Check sheet for the modelled part. Datum: model origin and axes. Units: mm. A direction names the side the tool comes from. Coordinates: 2 decimals unless noted, no trailing zeros. Write each loop counter-clockwise with the first axis right and the second up, starting at its lowest first coordinate (ties: lowest second). Pieces come first, ordered by that corner, then holes. Notation, with made-up numbers: (81, -8) -> (115, -8) arc R17 cw to (115, 3) -> close; hole circle Ø8 at (0, 4.5). An arc over 180 degrees is marked (long way). One line per item, written item: value. Start each with the question number.
1) Sectioned sample at A-A on x = -3. Enter the section's corners in (y, z).
2) Sectioned sample at B-B on y = 15.5. Enter the section's corners in (x, z).
3) Sectioned sample at D-D on y = -17.5. Enter the section's corners in (x, z).
4) Draft check along X on faces 5 (the flat face through (12, 23, 0)), 6 (the flat face through (0.18, -22.24, 6.92)), 7 (the flat face through (0, -21.5, 8)). Enter one of: +X half, -X half, draft (parallel to the pull), parting line (faces both ways), or undercut.
5) Scan lines: line 1 along Y through (x, z) = (1, 15); line 2 along Z through (x, y) = (0, 16); line 3 along Y through (x, z) = (-5.75, 10.75). Record each from-to range of solid material in increasing order. Write a range as [from, to].
6) Set-up check for faces 1 (the flat face through (0, 4, 3)), 2 (the flat face through (8.25, 16, -1)), 3 (the flat face through (0, -11, 14)), 4 (the cylindrical face through (10.288, -16.215, 5.296)): record each of +Z, -Z, +X, -X, +Y, -Y from which the full face is reachable in a straight line by a thin tool's end or side.
7) Gauge pin test, flat ends, axial feed: P1, Ø5, axis at x = -7.5, z = -0.5, coming from the -Y side; P2, Ø2, axis at x = 0, y = -17, coming from the -Z side; P3, Ø6, axis at x = -4.5, z = 12.5, coming from the +Y side; P4, Ø6.5, axis at x = 0, y = -18, coming from the -Z side. Record the tip position at first contact, or that the pin passes through.
8) Sectioned sample at C-C on z = 14. Enter the section's corners in (x, y), plus the area to 3 significant figures.
```python
from build123d import *

# Parameters (mm, degrees)
SKETCH1_W             = 25
SKETCH1_H             = 48
BOSS_EXTRUDE1_DEPTH   = 4
SKETCH5_W             = 25
SKETCH5_H             = 24
BOSS_EXTRUDE3_DEPTH   = 13
SKETCH6_W             = 20
SKETCH6_H             = 40
CUT_EXTRUDE1_DEPTH    = 1.5
M3_TAPPED_HOLE1_D     = 2.5
M3_TAPPED_HOLE1_DEPTH = 11.5
M3_TAPPED_HOLE1_TIP   = 0.751075774
CHAMFER2_SIZE         = 1.5
CUT_EXTRUDE3_DEPTH    = 37.169738733
SKETCH18_R            = 2
CUT_EXTRUDE5_DEPTH    = 1.5
CUT_EXTRUDE6_DEPTH    = 37.169738733
CUT_EXTRUDE7_DEPTH    = 41.012498047
CUT_EXTRUDE8_DEPTH    = 15
FILLET2_R             = 5
CHAMFER4_SIZE         = 0.5


with BuildPart() as part:
    # Sketch1 → Boss-Extrude1 (new, symmetric)
    with BuildSketch(Plane.XY):
        Rectangle(SKETCH1_W, SKETCH1_H)
    extrude(amount=BOSS_EXTRUDE1_DEPTH, both=True)

    # Sketch5 → Boss-Extrude3 (add)
    with BuildSketch(Plane.XZ.offset(24)):
        with Locations((0, 8)):
            Rectangle(SKETCH5_W, SKETCH5_H)
    extrude(amount=-BOSS_EXTRUDE3_DEPTH)

    # Sketch6 → Cut-Extrude1 (cut)
    with BuildSketch(Plane.XY.offset(4)):
        with Locations((0, 24)):
            Rectangle(SKETCH6_W, SKETCH6_H)
    extrude(amount=-CUT_EXTRUDE1_DEPTH, mode=Mode.SUBTRACT)

    # M3 Tapped Hole1
    with Locations(Plane(origin=(0, 24, 0), x_dir=(1, 0, 0), z_dir=(0, 1, 0))):
        with Locations((0, 2)):
            Hole(M3_TAPPED_HOLE1_D / 2, depth=M3_TAPPED_HOLE1_DEPTH)
            with Locations((0, 0, -(M3_TAPPED_HOLE1_DEPTH + M3_TAPPED_HOLE1_TIP / 2))):  # 118° drill point
                Cone(0, M3_TAPPED_HOLE1_D / 2, M3_TAPPED_HOLE1_TIP, mode=Mode.SUBTRACT)

    # Chamfer2
    chamfer2_edges = [part.edges().sort_by_distance(p)[0] for p in [
        (-12.5, 24, 0),
        (12.5, 24, 0),
    ]]
    chamfer(chamfer2_edges, length=CHAMFER2_SIZE)

    # Sketch14 → Cut-Extrude3 (cut, through all)
    with BuildSketch(Plane(origin=(0, 0, -4), x_dir=(-1, 0, 0), z_dir=(0, 0, -1))):
        with BuildLine():
            Line((-4.75, 19.5), (-4.75, 13.5))
            ThreePointArc((-4.75, 13.5), (-6.5, 11.75), (-8.25, 13.5))
            Line((-8.25, 13.5), (-8.25, 19.5))
            ThreePointArc((-8.25, 19.5), (-6.5, 21.25), (-4.75, 19.5))
        make_face()
        with BuildLine():
            Line((8.25, 19.5), (8.25, 13.5))
            ThreePointArc((8.25, 13.5), (6.5, 11.75), (4.75, 13.5))
            Line((4.75, 13.5), (4.75, 19.5))
            ThreePointArc((4.75, 19.5), (6.5, 21.25), (8.25, 19.5))
        make_face()
    extrude(amount=-CUT_EXTRUDE3_DEPTH, mode=Mode.SUBTRACT)

    # Sketch15 → M3 Tapped Hole2 (revolve, cut)
    with BuildSketch(Plane(origin=(-12.5, -9, 0), x_dir=(0, 0, 1), z_dir=(0, 1, 0))):
        Polygon((0, 0), (0, 12.251075774), (1.25, 11.5), (1.25, 0), align=None)
    m3_tapped_hole2 = revolve(axis=Axis((-18.85, -9, 0), (1, 0, 0)), mode=Mode.SUBTRACT)

    # Sketch18 → Cut-Extrude5 (cut)
    with BuildSketch(Plane.XY.offset(4)):
        with Locations((-8, 4)):
            Circle(SKETCH18_R)
        with Locations((8, 4)):
            Circle(SKETCH18_R)
    extrude(amount=-CUT_EXTRUDE5_DEPTH, mode=Mode.SUBTRACT)

    # Sketch20 → Cut-Extrude6 (cut, through all)
    with BuildSketch(Plane(origin=(0, 0, -4), x_dir=(-1, 0, 0), z_dir=(0, 0, -1))):
        with BuildLine():
            Line((-6.5, -15.25), (6.5, -15.25))
            ThreePointArc((6.5, -15.25), (8.75, -17.5), (6.5, -19.75))
            Line((6.5, -19.75), (-6.5, -19.75))
            ThreePointArc((-6.5, -19.75), (-8.75, -17.5), (-6.5, -15.25))
        make_face()
    extrude(amount=-CUT_EXTRUDE6_DEPTH, mode=Mode.SUBTRACT)

    # Sketch21 → Cut-Extrude7 (cut, through all)
    with BuildSketch(Plane(origin=(12.5, 0, 0), x_dir=(0, 0, -1), z_dir=(1, 0, 0))):
        Polygon((-9, -24), (4, -13), (4, -24), align=None)
    extrude(amount=-CUT_EXTRUDE7_DEPTH, mode=Mode.SUBTRACT)

    # Sketch22 → Cut-Extrude8 (cut)
    with BuildSketch(Plane(origin=(0, 0, -4), x_dir=(-1, 0, 0), z_dir=(0, 0, -1))):
        with BuildLine():
            Line((-6.5, -13.5), (6.5, -13.5))
            ThreePointArc((6.5, -13.5), (10.5, -17.5), (6.5, -21.5))
            Line((6.5, -21.5), (-6.5, -21.5))
            ThreePointArc((-6.5, -21.5), (-10.5, -17.5), (-6.5, -13.5))
        make_face()
    extrude(amount=-CUT_EXTRUDE8_DEPTH, mode=Mode.SUBTRACT)

    # Fillet2
    fillet2_edges = [part.edges().sort_by_distance(p)[0] for p in [
        (0, -11, 4),
    ]]
    fillet(fillet2_edges, radius=FILLET2_R)

    # Mirror1: M3 Tapped Hole2 across plane
    add(m3_tapped_hole2.mirror(Plane(origin=(0, 0, 0), x_dir=(0, 0, 1), z_dir=(1, 0, 0))), mode=Mode.SUBTRACT)

    # Chamfer4
    chamfer4_edges = [part.edges().sort_by_distance(p)[0] for p in [
        (0, -24, 20),
        (0, -11, 20),
    ]]
    chamfer(chamfer4_edges, length=CHAMFER4_SIZE)


solid = part.part
```
Answers:
1. outline: (-24, 9) -> (-21.5, 6.05) -> (-21.5, 11) -> (-19.75, 11) -> (-19.75, 20) -> (-23.5, 20) -> (-24, 19.5) -> close; (-15.25, 11) -> (-13.5, 11) -> (-13.5, -3.41) -> (-13, -4) -> (24, -4) -> (24, 2.5) -> (4, 2.5) -> (4, 4) -> (-6, 4) arc R5 cw to (-11, 9) -> (-11, 19.5) -> (-11.5, 20) -> (-15.25, 20) -> close; hole circle Ø2.5 at (-9, 0)
2. outline: (-12.5, -4) -> (-8.25, -4) -> (-8.25, 2.5) -> (-10, 2.5) -> (-10, 4) -> (-12.5, 4) -> close; (-4.75, -4) -> (4.75, -4) -> (4.75, 2.5) -> (-4.75, 2.5) -> close; (8.25, -4) -> (12.5, -4) -> (12.5, 4) -> (10, 4) -> (10, 2.5) -> (8.25, 2.5) -> close; hole circle Ø2.5 at (0, -2)
3. outline: (-12.5, 1.32) -> (-10.5, 1.32) -> (-10.5, 11) -> (-8.75, 11) -> (-8.75, 20) -> (-12.5, 20) -> close; (8.75, 11) -> (10.5, 11) -> (10.5, 1.32) -> (12.5, 1.32) -> (12.5, 20) -> (8.75, 20) -> close
4. face 5: +X half
4. face 6: draft
4. face 7: undercut
5. line 1: y = [-24, -19.75], [-15.25, -11]
5. line 2: z = [-4, -3.25], [-0.75, 2.5]
5. line 3: y = [-24, -21.5], [-13.5, -11]
6. face 1: +Z, +Y
6. face 2: +Z, -Z
6. face 3: +Z, +X, -X, +Y
6. face 4: -Z
7. P1: stops at y = -15.56
7. P2: passes through
7. P3: stops at y = -11
7. P4: stops at z = 11
8. outline: (-12.5, -24) -> (12.5, -24) -> (12.5, -11) -> (-12.5, -11) -> close; hole (-6.5, -19.75) -> (6.5, -19.75) arc R2.25 ccw to (6.5, -15.25) -> (-6.5, -15.25) arc R2.25 ccw to start
8. area: 251 mm2
